Source: CAD feature listing. Evaluate the final solid. Frame: model axes, mm. Face numbers are marked on the shaded views. Round coordinates to 2 decimals unless told otherwise and drop trailing zeros. Loops run counter-clockwise (first coordinate to the right, second up) from the corner with the lowest first, then second, coordinate; pieces in that order, holes last.
(1) Mould query, pull axis Z, two halves, no side actions, for the marked faces 1, 2 and 3. Classes: pulls with the +Z half, pulls with the -Z half, needs draft (parallel to the pull), parting line crosses it, or undercut.
(2) Section A-A, the plane z = 12.25. Return the cut outline in (x, y).
(3) Material intervals for probe 1 along X at (y, z) = (3.75, 12.5); probe 2 along Z at (x, y) = (30, 2.5); probe 3 along X at (y, z) = (5.5, 10), sorted ascending.
(4) Section B-B, the plane x = 30. Return the cut outline in (y, z), plus the area to 3 significant figures.
(5) Section C-C, the plane y = 3.5. Return the cut outline in (x, z), plus the area to 3 significant figures.
```python
from build123d import *

# Parameters (mm, degrees)
SKETCH1_W                  = 100
SKETCH1_H                  = 54.5
BOSS_EXTRUDE1_DEPTH        = 8
F_11_0_11_DIAMETER_HOLE1_D = 11


with BuildPart() as part:
    # Sketch1 → Boss-Extrude1 (new body)
    with BuildSketch(Plane(origin=(0, 0, 0), x_dir=(1, 0, 0), z_dir=(0, 1, 0))):
        Rectangle(SKETCH1_W, SKETCH1_H)
    extrude(amount=BOSS_EXTRUDE1_DEPTH)

    # Ø11.0 (11) Diameter Hole1 (through all)
    with Locations(Plane(origin=(0, 8, 0), x_dir=(1, 0, 0), z_dir=(0, 1, 0))):
        with Locations((-30, -12.25), (30, -12.25)):
            Hole(F_11_0_11_DIAMETER_HOLE1_D / 2)


solid = part.part
```
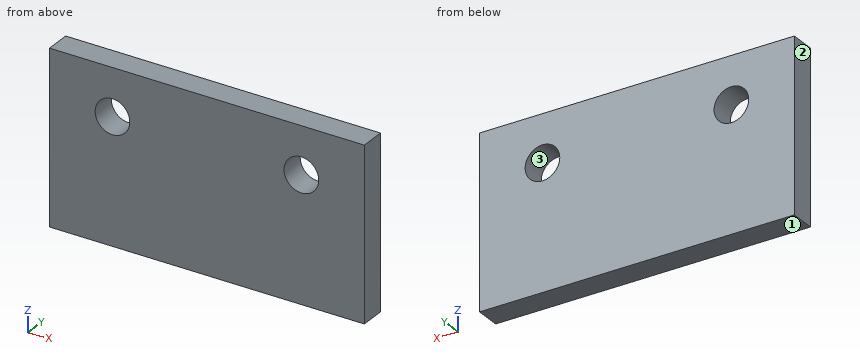
Output values:
1. face 1: pulls with the -Z half
1. face 2: needs draft
1. face 3: undercut
2. outline: (-50, 0) - (-35.5, 0) - (-35.5, 8) - (-50, 8) - close; (-24.5, 0) - (24.5, 0) - (24.5, 8) - (-24.5, 8) - close; (35.5, 0) - (50, 0) - (50, 8) - (35.5, 8) - close
3. probe 1: x = -50 to -35.49, -24.51 to 24.51, 35.49 to 50
3. probe 2: z = -27.25 to 6.75, 17.75 to 27.25
3. probe 3: x = -50 to -35.02, -24.98 to 24.98, 35.02 to 50
4. outline: (0, -27.25) - (8, -27.25) - (8, 6.75) - (0, 6.75) - close; (0, 17.75) - (8, 17.75) - (8, 27.25) - (0, 27.25) - close
4. area: 348 mm2
5. outline: (-50, -27.25) - (50, -27.25) - (50, 27.25) - (-50, 27.25) - close; hole circle Ø11 at (-30, 12.25); hole circle Ø11 at (30, 12.25)
5. area: 5,260 mm2
